Geometry: final body of the model. Coordinates: model frame, mm. A direction names the side the tool comes from. Give positions to 0.01 mm unless a question says otherwise; leave off trailing zeros. Write each loop counter-clockwise with the first axis right and the second up, starting at its lowest first coordinate (ties: lowest second). Pieces come first, ordered by that corner, then holes.
```python
from build123d import *

# Parameters (mm, degrees)
EXTRUDE_START       = 3
EXTRUDE_1_DEPTH     = 3
SKETCH_4_W          = 31
SKETCH_4_H          = 2
EXTRUDE_2_DEPTH     = 28
CUT_EXTRUDE_1_REACH = 58.285
SKETCH_5_R          = 3


with BuildPart() as part:
    # Sketch 1 → Revolve 1 (revolve)
    with BuildSketch(Plane.XY):
        Polygon((2, 16), (0, 16), (0, 0), (25, 0), (25, 16), (23, 16), (23, 9), (2, 9), align=None)
    revolve(axis=Axis((25, 0, 0), (-1, 0, 0)))

    # Sketch 2 → Extrude 1 (add)
    with BuildSketch(Plane.ZY.offset(EXTRUDE_START)):
        with BuildLine():
            Line((-16, 0), (-16, 24))
            Line((-16, 24), (16, 24))
            Line((16, 24), (16, 0))
            ThreePointArc((16, 0), (0, -16), (-16, 0))
        make_face()
    extrude_1 = extrude(amount=-EXTRUDE_1_DEPTH)

    # Mirror 1: Extrude 1 across plane
    add(extrude_1.mirror(Plane(origin=(12.5, 0, 0), x_dir=(0, 0, 1), z_dir=(1, 0, 0))))

    # Sketch 4 → Extrude 2 (add, symmetric)
    with BuildSketch(Plane.XY):
        with Locations((12.5, 23)):
            Rectangle(SKETCH_4_W, SKETCH_4_H)
    extrude(amount=EXTRUDE_2_DEPTH, both=True)

    # Sketch 5 → Cut-Extrude 1 (cut, up to next)
    with BuildSketch(Plane(origin=(0, 24, 0), x_dir=(1, 0, 0), z_dir=(0, 1, 0)), mode=Mode.PRIVATE) as cut_extrude_1_sk1:
        with Locations(Location((4, 21.5, 0), (0, 0, 180))):
            Circle(SKETCH_5_R)
    cut_extrude_1_tool1 = extrude(cut_extrude_1_sk1.sketch, amount=-CUT_EXTRUDE_1_REACH, mode=Mode.PRIVATE) & part.part
    # Sketch 5 → Cut-Extrude 1 (cut, up to next)
    with BuildSketch(Plane(origin=(0, 24, 0), x_dir=(1, 0, 0), z_dir=(0, 1, 0)), mode=Mode.PRIVATE) as cut_extrude_1_sk2:
        with Locations(Location((4, -21.5, 0), (0, 0, 270))):
            Circle(SKETCH_5_R)
    cut_extrude_1_tool2 = extrude(cut_extrude_1_sk2.sketch, amount=-CUT_EXTRUDE_1_REACH, mode=Mode.PRIVATE) & part.part
    # Sketch 5 → Cut-Extrude 1 (cut, up to next)
    with BuildSketch(Plane(origin=(0, 24, 0), x_dir=(1, 0, 0), z_dir=(0, 1, 0)), mode=Mode.PRIVATE) as cut_extrude_1_sk3:
        with Locations(Location((21, -21.5, 0), (0, 0, 180))):
            Circle(SKETCH_5_R)
    cut_extrude_1_tool3 = extrude(cut_extrude_1_sk3.sketch, amount=-CUT_EXTRUDE_1_REACH, mode=Mode.PRIVATE) & part.part
    # Sketch 5 → Cut-Extrude 1 (cut, up to next)
    with BuildSketch(Plane(origin=(0, 24, 0), x_dir=(1, 0, 0), z_dir=(0, 1, 0)), mode=Mode.PRIVATE) as cut_extrude_1_sk4:
        with Locations(Location((21, 21.5, 0), (0, 0, 270))):
            Circle(SKETCH_5_R)
    cut_extrude_1_tool4 = extrude(cut_extrude_1_sk4.sketch, amount=-CUT_EXTRUDE_1_REACH, mode=Mode.PRIVATE) & part.part
    add(cut_extrude_1_tool1.solids().sort_by_distance((4, 24, -21.5))[0], mode=Mode.SUBTRACT)
    add(cut_extrude_1_tool2.solids().sort_by_distance((4, 24, 21.5))[0], mode=Mode.SUBTRACT)
    add(cut_extrude_1_tool3.solids().sort_by_distance((21, 24, 21.5))[0], mode=Mode.SUBTRACT)
    add(cut_extrude_1_tool4.solids().sort_by_distance((21, 24, -21.5))[0], mode=Mode.SUBTRACT)


solid = part.part
```
Item 1: Section A-A, the plane y = 19.5. Return the cut outline in (x, z).
Found:
outline: (-3, -16) - (0, -16) - (0, 16) - (-3, 16) - close; (25, -16) - (28, -16) - (28, 16) - (25, 16) - close
Item 2: Section C-C, the plane z = -21.5. Return the cut outline in (x, y).
Found:
outline: (-3, 22) - (1, 22) - (1, 24) - (-3, 24) - close; (7, 22) - (18, 22) - (18, 24) - (7, 24) - close; (24, 22) - (28, 22) - (28, 24) - (24, 24) - close
Item 3: Section B-B, the plane x = 4. Return the cut outline in (y, z), plus the area to 3 significant figures.
Found:
outline: circle Ø18 at (0, 0); (22, -28) - (24, -28) - (24, -24.5) - (22, -24.5) - close; (22, -18.5) - (24, -18.5) - (24, 18.5) - (22, 18.5) - close; (22, 24.5) - (24, 24.5) - (24, 28) - (22, 28) - close
area: 342 mm2
Item 4: Pull-direction query (Y, two-part tool) for faces 4 (the face through (28, 4, 0)), 5 (the face through (12, 22, 0)), 6 (the face through (12, 24, 0)); classes: +Y half, -Y half, draft (parallel to the pull), parting line (faces both ways), or undercut.
Found:
face 4: draft
face 5: undercut
face 6: +Y half
Item 5: Section D-D, the plane x = 14. Return the cut outline in (y, z).
Found:
outline: circle Ø18 at (0, 0); (22, -28) - (24, -28) - (24, 28) - (22, 28) - close
Item 6: Reachability of faces 1 (the face through (2, -7, 7)), 2 (the face through (27, 11, -16)), 3 (the face through (27, 11, 16)) from +Z, -Z, +X, -X, +Y, -Y: full face, straight path, thin tool, end or side. Return the list, or none.
Found:
face 1: none
face 2: -Z, +X, -X, -Y
face 3: +Z, +X, -X, -Y
Item 7: Line query: L1, parallel to Z at x = -1.5, y = -0.5; L2, parallel to Y at x = 11, z = -21.5; L3, parallel to Z at x = 23, y = 22.5. Output: solid intervals per line, ascending.
Found:
L1: z = -15.99 to 15.99
L2: y = 22 to 24
L3: z = -28 to -23.74, -19.26 to 19.26, 23.74 to 28
Item 8: Pin query (flat end, axial travel): pin 1 Ø5 at (x, z) = (19, 17.5) entering from -Y; pin 2 Ø0.9 at (x, y) = (-1, 14) entering from -Z; pin 3 Ø12 at (x, y) = (9.5, -9) entering from +Z. Return the tip coordinate at first contact, or that it passes through.
Found:
pin 1: stops at y = 22
pin 2: stops at z = -16
pin 3: stops at z = 8.49
